Read the model definition and answer for the solid it produces. Units are mm, in the model's axes. Give positions to 0.01 mm unless a question says otherwise; leave off trailing zeros. Order: outer loops, then holes, each group sorted by start corner. A loop starts at its lowest first (then second) coordinate and runs counter-clockwise, first axis right, second up. Notation, with made-up numbers: (-37, 51.25) -> (-6, 51.25) arc R17 ccw to (-6, 60.25) -> close; hole circle Ø5 at (-21, 37.5). An arc over 180 degrees is marked (long way). Use one line per item in the form item = value.
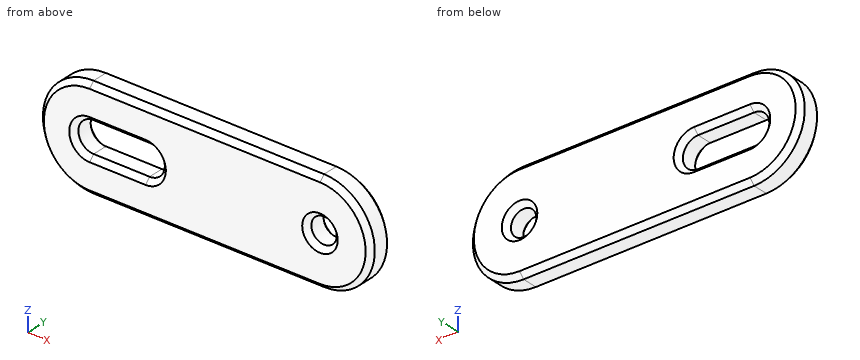
```python
from build123d import *

# Parameters (mm, degrees)
SKETCH1_R           = 2.5
BOSS_EXTRUDE1_DEPTH = 5
CHAMFER1_SIZE       = 1


with BuildPart() as part:
    # Sketch1 → Boss-Extrude1 (new body)
    with BuildSketch(Plane(origin=(0, 0, 0), x_dir=(1, 0, 0), z_dir=(0, 1, 0))):
        with BuildLine():
            Line((0, -10), (-45.398085341, -10))
            ThreePointArc((-45.398085341, -10), (-55.398085341, 0), (-45.398085341, 10))
            Line((-45.398085341, 10), (0, 10))
            ThreePointArc((0, 10), (10, 0), (0, -10))
        make_face()
        with Locations(Location((0, 0, 0), (0, 0, 270))):
            Circle(SKETCH1_R, mode=Mode.SUBTRACT)
        with BuildLine():
            Line((-45.398085341, 3), (-34.372756479, 3))
            ThreePointArc((-34.372756479, 3), (-31.372756479, 0), (-34.372756479, -3))
            Line((-34.372756479, -3), (-45.398085341, -3))
            ThreePointArc((-45.398085341, -3), (-48.398085341, 0), (-45.398085341, 3))
        make_face(mode=Mode.SUBTRACT)
    extrude(amount=BOSS_EXTRUDE1_DEPTH)

    # Chamfer1
    chamfer1_edges = [part.edges().sort_by_distance(p)[0] for p in [
        (0, 0, -2.5),
        (0, 5, -2.5),
        (-55.398085341, 5, 0),
        (-22.69904267, 5, 10),
        (-48.398085341, 0, 0),
        (-39.88542091, 0, 3),
        (-31.372756479, 0, 0),
        (-39.88542091, 0, -3),
        (-48.398085341, 5, 0),
        (-39.88542091, 5, 3),
        (-31.372756479, 5, 0),
        (-39.88542091, 5, -3),
        (10, 5, 0),
        (-22.69904267, 0, 10),
        (-55.398085341, 0, 0),
        (-22.69904267, 0, -10),
        (10, 0, 0),
        (-22.69904267, 5, -10),
    ]]
    chamfer(chamfer1_edges, length=CHAMFER1_SIZE)


solid = part.part
```
Item 1: The part is cut by section C-C on y = 1.55. Give the vertices of the cut face in (x, z).
Checks:
outline = (-45.4, -10) -> (0, -10) arc R10 ccw to (0, 10) -> (-45.4, 10) arc R10 ccw to start; hole (-45.4, -3) -> (-34.37, -3) arc R3 ccw to (-34.37, 3) -> (-45.4, 3) arc R3 ccw to start; hole circle Ø5 at (0, 0)
Item 2: The part is cut by section B-B on z = 0. Give the vertices of the cut face in (x, y).
Checks:
outline = (-55.4, 1) -> (-54.4, 0) -> (-49.4, 0) -> (-48.4, 1) -> (-48.4, 4) -> (-49.4, 5) -> (-54.4, 5) -> (-55.4, 4) -> close; (-31.37, 1) -> (-30.37, 0) -> (-3.5, 0) -> (-2.5, 1) -> (-2.5, 4) -> (-3.5, 5) -> (-30.37, 5) -> (-31.37, 4) -> close; (2.5, 1) -> (3.5, 0) -> (9, 0) -> (10, 1) -> (10, 4) -> (9, 5) -> (3.5, 5) -> (2.5, 4) -> close
Item 3: The part is cut by section A-A on x = -43. Give the vertices of the cut face in (y, z), and give its area (3 significant figures).
Checks:
outline = (0, -9) -> (1, -10) -> (4, -10) -> (5, -9) -> (5, -4) -> (4, -3) -> (1, -3) -> (0, -4) -> close; (0, 4) -> (1, 3) -> (4, 3) -> (5, 4) -> (5, 9) -> (4, 10) -> (1, 10) -> (0, 9) -> close
area = 66.0 mm²
Item 4: The part is cut by section D-D on x = -9.5. Give the vertices of the cut face in (y, z), and give its area (3 significant figures).
Checks:
outline = (0, -9) -> (1, -10) -> (4, -10) -> (5, -9) -> (5, 9) -> (4, 10) -> (1, 10) -> (0, 9) -> close
area = 98.0 mm²
Item 5: Straight lines are drawn through the part: L1, parallel to X at y = 3.3, z = 0; L2, parallel to X at y = 4.6, z = 0.5; L3, parallel to Z at x = -44.5, y = 1.1. For each, find the intervals that lie inside material, in ascending order. Write a range as from..to.
Checks:
L1 = -55.4..-48.4, -31.37..-2.5, 2.5..10
L2 = -54.78..-48.96, -30.81..-3.06, 3.06..9.39
L3 = -10..-3, 3..10
